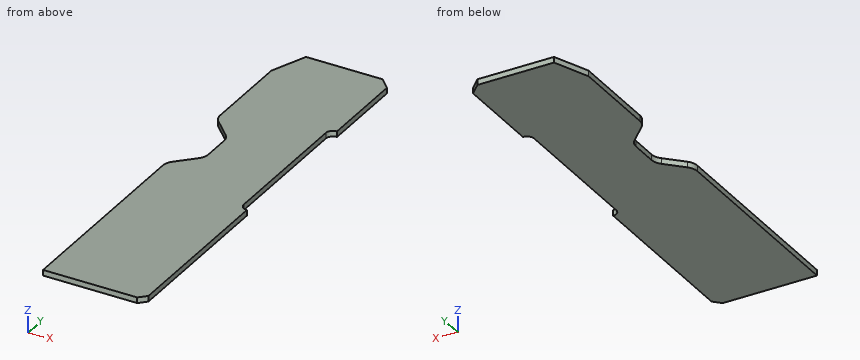
from build123d import *

# Parameters (mm, degrees)
BOSS_EXTRUDE1_DEPTH = 8


with BuildPart() as part:
    # Sketch1 → Boss-Extrude1 (new body)
    with BuildSketch(Plane.XY):
        with BuildLine():
            Line((0, 0), (0, 291.715728753))
            ThreePointArc((0, 291.715728753), (1.52240935, 299.3693974), (5.857864376, 305.857864376))
            Line((5.857864376, 305.857864376), (29.142135624, 329.142135624))
            ThreePointArc((29.142135624, 329.142135624), (33.47759065, 335.6306026), (35, 343.284271247))
            Line((35, 343.284271247), (35, 380.715728753))
            ThreePointArc((35, 380.715728753), (33.47759065, 388.3693974), (29.142135624, 394.857864376))
            Line((29.142135624, 394.857864376), (5.857864376, 418.142135624))
            ThreePointArc((5.857864376, 418.142135624), (1.52240935, 424.6306026), (0, 432.284271247))
            Line((0, 432.284271247), (0, 557))
            Line((0, 557), (20, 607))
            Line((20, 607), (128, 607))
            Line((128, 607), (143, 592))
            Line((143, 592), (143, 470))
            ThreePointArc((143, 470), (135.928932188, 467.071067812), (133, 460))
            Line((133, 460), (133, 260))
            ThreePointArc((133, 260), (135.928932188, 252.928932188), (143, 250))
            Line((143, 250), (143, 10))
            Line((143, 10), (133, 0))
            Line((133, 0), (0, 0))
        make_face()
    extrude(amount=BOSS_EXTRUDE1_DEPTH)


solid = part.part
Geometry: final body of the model. Coordinates: model frame, mm. Round coordinates to 2 decimals unless told otherwise and drop trailing zeros. Order: outer loops, then holes, each group sorted by start corner. A loop starts at its lowest first (then second) coordinate and runs counter-clockwise, first axis right, second up. Notation, with made-up numbers: (28, -18) -> (38, -18) arc R21 cw to (38, 18) -> close; hole circle Ø3 at (41.25, 32.25). An arc over 180 degrees is marked (long way). Put each result on its own line as item: value. Start each with the question number.
Q1. First-contact query: pin 1 (10 mm diameter, centred on x = 52.5, y = 361, fed in from -Z). Flat tip, straight axial feed; report the tip coordinate or a pass-through.
Q2. Section B-B on x = 14. Return the cut outline in (y, z).
Q3. Section D-D on y = 274. Return the cut outline in (x, z), and give its area (3 significant figures).
Q4. Line query: probe 1 along X at (y, z) = (372.5, 5); probe 2 along X at (y, z) = (265.5, 6); probe 3 along Y at (x, z) = (131.5, 5.25). Output: solid intervals per line, ascending.
Q5. Section C-C on y = 371.5. Return the cut outline in (x, z), and give its area (3 significant figures).
Q6. Section A-A on z = 3.25. Return the cut outline in (x, y), and give its area (3 significant figures).
Ans:
1. pin 1: stops at z = 0
2. outline: (0, 0) -> (314, 0) -> (314, 8) -> (0, 8) -> close; (410, 0) -> (592, 0) -> (592, 8) -> (410, 8) -> close
3. outline: (0, 0) -> (133, 0) -> (133, 8) -> (0, 8) -> close
3. area: 1,060 mm2
4. probe 1: x = 35 to 133
4. probe 2: x = 0 to 133
4. probe 3: y = 0 to 603.5
5. outline: (35, 0) -> (133, 0) -> (133, 8) -> (35, 8) -> close
5. area: 784 mm2
6. outline: (0, 0) -> (133, 0) -> (143, 10) -> (143, 250) arc R10 cw to (133, 260) -> (133, 460) arc R10 cw to (143, 470) -> (143, 592) -> (128, 607) -> (20, 607) -> (0, 557) -> (0, 432.28) arc R20 ccw to (5.86, 418.14) -> (29.14, 394.86) arc R20 cw to (35, 380.72) -> (35, 343.28) arc R20 cw to (29.14, 329.14) -> (5.86, 305.86) arc R20 ccw to (0, 291.72) -> close
6. area: 80,900 mm2
